Design review of the part built by this model. Coordinates are the model's own, in mm. A direction names the side the tool comes from. Give positions to 0.01 mm unless a question says otherwise; leave off trailing zeros. Write each loop counter-clockwise with the first axis right and the second up, starting at its lowest first coordinate (ties: lowest second). Pieces come first, ordered by that corner, then holes. Notation, with made-up numbers: M -32,-26 L 2,-26 A21 cw 2,-18 Z; hole C 52,-37.5 d11. An arc over 180 degrees is marked long. Use one line per item in the form item = value. Start each with the question number.
from build123d import *

# Parameters (mm, degrees)
BASE_EXTRUDE_DEPTH      = 6.4
FILLET_2_R              = 0.4
CUT_EXTRUDE1_DEPTH      = 23.928003257
CUT_EXTRUDE1_DEPTH_BACK = 23.928003257
SKETCH8_W               = 2.9
SKETCH8_H               = 16


with BuildPart() as part:
    # Sketch1 → Base-Extrude (new body)
    with BuildSketch(Plane(origin=(0, 0, 0), x_dir=(0, 0, -1), z_dir=(1, 0, 0))):
        Polygon((8, 4.618802154), (8, -4.618802154), (0, -9.237604307), (-8, -4.618802154), (-8, 4.618802154), (0, 9.237604307), align=None)
    extrude(amount=BASE_EXTRUDE_DEPTH)

    # Sketch2 → Boss-Revolve1 (revolve)
    with BuildSketch(Plane.XY, mode=Mode.PRIVATE) as boss_revolve1_sk:
        Polygon((0, 0), (32.4, 0), (32.4, 4.134), (32.4, 5), (27.8072, 5), (0, 5), align=None)
    revolve(boss_revolve1_sk.sketch.rotate(Axis((0, 0, 0), (1, 0, 0)), 90), axis=Axis((0, 0, 0), (1, 0, 0)))

    # Sketch3 → Cut-Revolve1 (revolve, cut)
    with BuildSketch(Plane.XY):
        Polygon((0, 8), (3.601282526, 14.237604307), (3.601282526, 19.237604307), (-10, 19.237604307), (-10, 8), align=None)
    revolve(axis=Axis((0, 0, 0), (1, 0, 0)), mode=Mode.SUBTRACT)

    # Fillet 2
    fillet_2_edges = [part.edges().sort_by_distance(p)[0] for p in [
        (6.4, 0, -5),
    ]]
    fillet(fillet_2_edges, radius=FILLET_2_R)

    # Sketch7 → Cut-Revolve5 (revolve, cut)
    with BuildSketch(Plane(origin=(0, 0, 0), x_dir=(1, 0, 0), z_dir=(0, 1, 0))):
        Polygon((32.4, 5), (18.4, 5), (19.4, 4), (19.4, 0), (32.4, 0), align=None)
    revolve(axis=Axis((34.209458749, 0, 0), (-1, 0, 0)), mode=Mode.SUBTRACT)

    # Sketch8 → Cut-Extrude1 (cut, two sides: drawn at the far end of the back side and taken through both)
    with BuildSketch(Plane(origin=(0, 0, 0), x_dir=(1, 0, 0), z_dir=(0, 1, 0)).offset(-CUT_EXTRUDE1_DEPTH_BACK)):
        with Locations((1.45, 0)):
            Rectangle(SKETCH8_W, SKETCH8_H)
    extrude(amount=CUT_EXTRUDE1_DEPTH + CUT_EXTRUDE1_DEPTH_BACK, mode=Mode.SUBTRACT)

    # Sketch9 → Revolve1 (revolve)
    with BuildSketch(Plane(origin=(0, 0, 0), x_dir=(1, 0, 0), z_dir=(0, 1, 0))):
        with BuildLine():
            Line((-5.1, 0), (-5.1, 2.5))
            ThreePointArc((-5.1, 2.5), (-1.393005283, 3.038009057), (0.9, 6))
            Line((0.9, 6), (0.9, 7))
            Line((0.9, 7), (2.9, 7))
            Line((2.9, 7), (2.9, 0))
            Line((2.9, 0), (-5.1, 0))
        make_face()
    revolve(axis=Axis((-7.317514451, 0, 0), (1, 0, 0)))

    # Sketch10 → Cut-Revolve6 (revolve, cut)
    with BuildSketch(Plane(origin=(0, 0, 0), x_dir=(1, 0, 0), z_dir=(0, 1, 0)), mode=Mode.PRIVATE) as cut_revolve6_sk:
        with BuildLine():
            Line((19.4, 0), (19.4, 2))
            Line((19.4, 2), (-0.22471637, 2))
            Line((-0.22471637, 2), (-0.22471637, 1.5))
            Line((-0.22471637, 1.5), (-4.1, 1.5))
            ThreePointArc((-4.1, 1.5), (-4.635233135, 1.401258538), (-5.1, 1.118033989))
            Line((-5.1, 1.118033989), (-5.1, 0))
            Line((-5.1, 0), (19.4, 0))
        make_face()
    revolve(cut_revolve6_sk.sketch.rotate(Axis((-5.799172577, 0, 0), (1, 0, 0)), 180), axis=Axis((-5.799172577, 0, 0), (1, 0, 0)), mode=Mode.SUBTRACT)


solid = part.part
1. We need section D-D (x = 0.5). State the section outline as (y, z) points, and give its area (3 significant figures).
2. We need section A-A (x = 3.25). State the section outline as (y, z) points, and give its area (3 significant figures).
3. For faces 1 (the flat face through (2.9, 7, 2)), 2 (the cylindrical face through (13, 0, -5)), 3 (the flat face through (-5.1, -1, 1)), list the 3-axis set-ups (+Z, -Z, +X, -X, +Y, -Y) from which the entire face can be reached by the end or side of a thin tool; tool diameter is ignored.
4. We need section C-C (y = 6.5). State the section outline as (x, z) points, and give its area (3 significant figures).
5. Clearance check with flat-ended pins moving along their axes: pin 1 Ø3 at (x, z) = (3.5, 6) entering from +Y; pin 2 Ø1.5 at (y, z) = (-4.5, -1.5) entering from -X; pin 3 Ø1 at (x, z) = (14.5, -6) entering from -Y; pin 4 Ø4 at (x, z) = (16, 3) entering from -Y. State where each tip first meets the part, or that it passes through.
6. To check wall thickness, follow L1, parallel to X at y = 7.25, z = 0.25; L2, parallel to Y at x = -2.85, z = 0; L3, parallel to Y at x = -1.1, z = 0. State the ranges of each line that lie inside material, in increasing order.
7. Draft analysis for pull direction Y (two halves, no side actions). For faces 4 (the flat face through (19.4, 1, 2)), 5 (the flat face through (4.626, -6.896, -4.056)), 6 (the cylindrical face through (9, 2, 0)), state which applies: pulls with the +Y half, pulls with the -Y half, needs draft (parallel to the pull), parting line crosses it, or undercut.
Answer block:
q1.outline = C 0,0 d10.01; hole C 0,0 d4
q1.area = 66.1 mm^2
q2.outline = M -9.24,0 L -4.62,-8 L 4.62,-8 L 9.24,0 L 4.62,8 L -4.62,8 Z; hole C 0,0 d4
q2.area = 209 mm^2
q3.face_1 = -X
q3.face_2 = +X
q3.face_3 = +Z, -Z, -X, +Y, -Y
q4.outline = M 0.9,-2.6 L 2.9,-2.6 L 2.9,-4.74 L 6.4,-4.74 L 6.4,4.74 L 2.9,4.74 L 2.9,2.6 L 0.9,2.6 Z
q4.area = 43.6 mm^2
q5.pin_1 = 6.64
q5.pin_2 = -0.21
q5.pin_3 = through
q5.pin_4 = -4.9
q6.L1 = 2.9 to 6.4
q6.L2 = -2.47 to -1.5, 1.5 to 2.47
q6.L3 = -3.22 to -1.5, 1.5 to 3.22
q7.face_4 = needs draft
q7.face_5 = pulls with the -Y half
q7.face_6 = undercut
